Read the model definition and answer for the solid it produces. Units are mm, in the model's axes. Face numbers are marked on the shaded views. A direction names the side the tool comes from. Round coordinates to 2 decimals unless told otherwise and drop trailing zeros. Write each loop counter-clockwise with the first axis right and the second up, starting at its lowest first coordinate (ties: lowest second). Pieces come first, ordered by that corner, then holes. Notation, with made-up numbers: (69.25, 43.25) - (89.25, 43.25) arc R20 cw to (89.25, 58.25) - close; hole circle Ø11 at (31, 42). An arc over 180 degrees is marked (long way). Answer as CSV lines item,"result". Start each with the question number.
1) Consider line 1 along Z through (x, y) = (72.5, 5); line 2 along X through (y, z) = (44, 41). Determine where each line is inside the solid, lowest interval first.
2) Each of these flat-tipped pins is pushed along its axis until it touches: pin 1 (1.5 mm diameter, centred on x = 24.5, z = 2, fed in from +Y); pin 2 (3 mm diameter, centred on y = 17.5, z = 21.5, fed in from +X). Where does it stop, or does it pass through?
3) Find section B-B on x = 75.5. Determine the outline of the cut face in (y, z), then the cut area to 3 significant figures.
4) Which of the six approach directions +Z, -Z, +X, -X, +Y, -Y give full straight-line access (tool end or side, diameter ignored) to the marked faces 1 and 2?
5) Find section A-A on z = 0. Determine the outline of the cut face in (x, y), then the cut area to 3 significant figures.
6) Find section C-C on y = 16. Determine the outline of the cut face in (x, z), then the cut area to 3 significant figures.
7) Find section D-D on x = 88. Determine the outline of the cut face in (y, z).
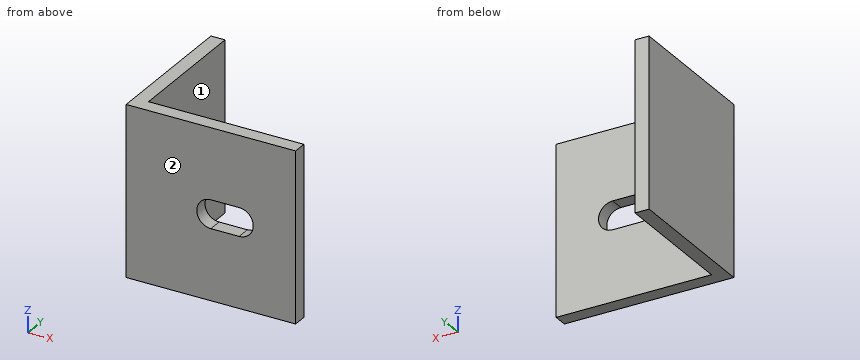
from build123d import *

# Parameters (mm, degrees)
EXTRUDE_THIN1_DEPTH = 60
CUT_EXTRUDE1_DEPTH  = 164.245214325


with BuildPart() as part:
    # Sketch1 → Extrude-Thin1 (new, symmetric)
    with BuildSketch(Plane.XY):
        Polygon((120, 0), (0, 0), (0, 103), (10, 103), (10, 10), (120, 10), align=None)
    extrude(amount=EXTRUDE_THIN1_DEPTH, both=True)

    # Sketch2 → Cut-Extrude1 (cut, through all)
    with BuildSketch(Plane(origin=(0, 10, 0), x_dir=(1, 0, 0), z_dir=(0, 1, 0))):
        with BuildLine():
            Line((60, 10), (80, 10))
            ThreePointArc((80, 10), (90, 0), (80, -10))
            Line((80, -10), (60, -10))
            ThreePointArc((60, -10), (50, 0), (60, 10))
        make_face()
    extrude(amount=-CUT_EXTRUDE1_DEPTH, mode=Mode.SUBTRACT)


solid = part.part
Check values:
1,line 1,"z = -60 to -10, 10 to 60"
1,line 2,"x = 0 to 10"
2,pin 1,"stops at y = 10"
2,pin 2,"stops at x = 10"
3,outline,"(0, -60) - (10, -60) - (10, -10) - (0, -10) - close; (0, 10) - (10, 10) - (10, 60) - (0, 60) - close"
3,area,"1,000 mm^2"
4,face 1,"+Z, -Z, +X, +Y"
4,face 2,"+Z, -Z, +X, -X, -Y"
5,outline,"(0, 0) - (50, 0) - (50, 10) - (10, 10) - (10, 103) - (0, 103) - close; (90, 0) - (120, 0) - (120, 10) - (90, 10) - close"
5,area,"1,730 mm^2"
6,outline,"(0, -60) - (10, -60) - (10, 60) - (0, 60) - close"
6,area,"1,200 mm^2"
7,outline,"(0, -60) - (10, -60) - (10, -6) - (0, -6) - close; (0, 6) - (10, 6) - (10, 60) - (0, 60) - close"
